```python
from build123d import *

# Parameters (mm, degrees)
LEVER_PLATE_16MM_DEPTH     = 16
HUB_FRONT_SKETCH_35_R      = 17.5
HUB_FRONT_BOSS_35X13_DEPTH = 13
HUB_START                  = 3
HUB_BACK_SKETCH_35_R       = 17.5
HUB_BACK_BOSS_35X3_DEPTH   = 3
KEYED_BORE_CUT_DEPTH       = 60
SLOT_RIM_A_2MM_DEPTH       = 2
SLOT_START                 = 2
SLOT_RIM_B_2MM_DEPTH       = 2


with BuildPart() as part:
    # Lever Profile Sketch → Lever Plate 16mm (new body)
    with BuildSketch(Plane.XY):
        with BuildLine():
            ThreePointArc((101.261586429, -17.5), (112.844778282, -11.952124129), (117.545415365, 0))
            ThreePointArc((117.545415365, 0), (113.540152463, 30.422992161), (101.797315804, 58.772707682))
            ThreePointArc((101.797315804, 58.772707682), (88.2863604, 67.464431009), (73.363703567, 61.514113087))
            ThreePointArc((73.363703567, 61.514113087), (37.333335855, 34.13389002), (-4.513207912, 16.9080145))
            ThreePointArc((-4.513207912, 16.9080145), (-17.351372478, -2.275933462), (0, -17.5))
            Line((0, -17.5), (101.261586429, -17.5))
        make_face()
        with BuildLine():
            ThreePointArc((71.407764953, 41.227292318), (79.645012795, 21.34081686), (82.454584635, 0))
            ThreePointArc((82.454584635, 0), (83.56318735, -6.137816406), (86.74890192, -11.5))
            Line((86.74890192, -11.5), (42.586205582, -11.5))
            ThreePointArc((42.586205582, -11.5), (23.157647429, 3.753303456), (33.364058597, 26.246887192))
            ThreePointArc((33.364058597, 26.246887192), (51.952476434, 37.375508628), (69.069413247, 50.656546497))
            ThreePointArc((69.069413247, 50.656546497), (69.572959936, 45.776850669), (71.407764953, 41.227292318))
        make_face(mode=Mode.SUBTRACT)
        with BuildLine():
            ThreePointArc((91.25, 0), (88.140731649, 23.617237866), (79.024818095, 45.625))
            ThreePointArc((79.024818095, 45.625), (82.227540378, 57.577722283), (94.180262662, 54.375))
            ThreePointArc((94.180262662, 54.375), (105.044433609, 28.146571155), (108.75, 0))
            ThreePointArc((108.75, 0), (100, -8.75), (91.25, 0))
        make_face(mode=Mode.SUBTRACT)
    extrude(amount=LEVER_PLATE_16MM_DEPTH)

    # Hub Front Sketch Ø35 → Hub Front Boss Ø35x13 (add)
    with BuildSketch(Plane.XY.offset(16)):
        with Locations(Location((0, 0, 0), (0, 0, 104.94534936))):
            Circle(HUB_FRONT_SKETCH_35_R)
    extrude(amount=HUB_FRONT_BOSS_35X13_DEPTH)

    # Hub Back Sketch Ø35 → Hub Back Boss Ø35x3 (add)
    with BuildSketch(Plane(origin=(0, 0, 0), x_dir=(-1, 0, 0), z_dir=(0, 0, -1)).offset(HUB_START)):
        Circle(HUB_BACK_SKETCH_35_R)
    extrude(amount=-HUB_BACK_BOSS_35X3_DEPTH)

    # Keyed Bore Sketch → Keyed Bore Cut (cut)
    with BuildSketch(Plane.XY.offset(29)):
        with BuildLine():
            ThreePointArc((-10.583005244, -3), (1.514421063, -10.895252583), (11, 0))
            Line((11, 0), (-13.5, 0))
            Line((-13.5, 0), (-13.5, -3))
            Line((-13.5, -3), (-10.583005244, -3))
        make_face()
        with BuildLine():
            Line((-13.5, 0), (11, 0))
            ThreePointArc((11, 0), (1.514421063, 10.895252583), (-10.583005244, 3))
            Line((-10.583005244, 3), (-13.5, 3))
            Line((-13.5, 3), (-13.5, 0))
        make_face()
    extrude(amount=-KEYED_BORE_CUT_DEPTH, mode=Mode.SUBTRACT)

    # Slot Rim Sketch A → Slot Rim A 2mm (add)
    with BuildSketch(Plane.XY.offset(16)):
        with BuildLine():
            ThreePointArc((117.545415365, 0), (113.540152463, 30.422992161), (101.797315804, 58.772707682))
            ThreePointArc((101.797315804, 58.772707682), (77.829832696, 65.194775426), (71.407764953, 41.227292318))
            ThreePointArc((71.407764953, 41.227292318), (79.645012795, 21.34081686), (82.454584635, 0))
            ThreePointArc((82.454584635, 0), (100, -17.545415365), (117.545415365, 0))
        make_face()
        with BuildLine():
            ThreePointArc((108.75, 0), (105.044433609, 28.146571155), (94.180262662, 54.375))
            ThreePointArc((94.180262662, 54.375), (82.227540378, 57.577722283), (79.024818095, 45.625))
            ThreePointArc((79.024818095, 45.625), (88.140731649, 23.617237866), (91.25, 0))
            ThreePointArc((91.25, 0), (100, -8.75), (108.75, 0))
        make_face(mode=Mode.SUBTRACT)
    extrude(amount=SLOT_RIM_A_2MM_DEPTH)

    # Slot Rim Sketch B → Slot Rim B 2mm (add)
    with BuildSketch(Plane(origin=(0, 0, 0), x_dir=(-1, 0, 0), z_dir=(0, 0, -1)).offset(SLOT_START)):
        with BuildLine():
            ThreePointArc((-101.797315804, 58.772707682), (-113.540152463, 30.422992161), (-117.545415365, 0))
            ThreePointArc((-117.545415365, 0), (-100, -17.545415365), (-82.454584635, 0))
            ThreePointArc((-82.454584635, 0), (-79.645012795, 21.34081686), (-71.407764953, 41.227292318))
            ThreePointArc((-71.407764953, 41.227292318), (-77.829832696, 65.194775426), (-101.797315804, 58.772707682))
        make_face()
        with BuildLine():
            ThreePointArc((-94.180262662, 54.375), (-105.044433609, 28.146571155), (-108.75, 0))
            ThreePointArc((-108.75, 0), (-100, -8.75), (-91.25, 0))
            ThreePointArc((-91.25, 0), (-88.140731649, 23.617237866), (-79.024818095, 45.625))
            ThreePointArc((-79.024818095, 45.625), (-82.227540378, 57.577722283), (-94.180262662, 54.375))
        make_face(mode=Mode.SUBTRACT)
    extrude(amount=-SLOT_RIM_B_2MM_DEPTH)


solid = part.part
```
Input: part model. Units: mm. Frame: model coordinates. A direction names the side the tool comes from. Coordinates: 2 decimals unless noted, no trailing zeros. Write each loop counter-clockwise with the first axis right and the second up, starting at its lowest first coordinate (ties: lowest second). Pieces come first, ordered by that corner, then holes. Notation, with made-up numbers: (64.5, 67.5) -> (96.5, 67.5) arc R4 cw to (96.5, 72.5) -> close; hole circle Ø9 at (9, -30.75). An arc over 180 degrees is marked (long way). Answer as a JSON object with one key per item and string values.
1. Section D-D on y = -4.5. Return the cut outline in (x, z), then the cut area to 3 significant figures.
Result set:
{"outline": "(-16.91, -3) -> (-10.04, -3) -> (-10.04, 29) -> (-16.91, 29) -> close; (10.04, -3) -> (16.91, -3) -> (16.91, 0) -> (27.39, 0) -> (27.39, 16) -> (16.91, 16) -> (16.91, 29) -> (10.04, 29) -> close; (83.04, -2) -> (92.5, -2) -> (92.5, 18) -> (83.04, 18) -> close; (107.5, -2) -> (116.96, -2) -> (116.96, 18) -> (107.5, 18) -> close", "area": "986 mm2"}
2. Section B-B on y = 48. Return the cut outline in (x, z).
Result set:
{"outline": "(57.98, 0) -> (65.97, 0) -> (65.97, 16) -> (57.98, 16) -> close; (69.17, -2) -> (78.08, -2) -> (78.08, 18) -> (69.17, 18) -> close; (97.58, -2) -> (107.3, -2) -> (107.3, 18) -> (97.58, 18) -> close"}
3. Section C-C on x = 41. Return the cut outline in (y, z).
Result set:
{"outline": "(-17.5, 0) -> (-11.44, 0) -> (-11.44, 16) -> (-17.5, 16) -> close; (30.45, 0) -> (36.29, 0) -> (36.29, 16) -> (30.45, 16) -> close"}
4. First-contact query: P1, Ø2, axis at y = 14.5, z = 22.5, coming from the -X side; P2, Ø13, axis at x = 75, z = 8.5, coming from the +Y side; P3, Ø4, axis at y = 10, z = 15, coming from the -X side. Flat tips, straight axial feed; report the tip coordinate or a pass-through.
Result set:
{"P1": "stops at x = -11.14", "P2": "stops at y = 66.79", "P3": "stops at x = -15.56"}
5. Access query for faces 1 (the face through (-12, 3, 13)), 2 (the face through (88, 16, 18)), 3 (the face through (24, -1, 0)), 4 (the face through (113.428, 30.839, 7.86)). Directions: +Z, -Z, +X, -X, +Y, -Y. A direction counts if a zero-diameter tool reaches every point of the face in a straight line with its end or side. Return the directions, or none.
Result set:
{"face 1": "+Z, -Z", "face 2": "+Z, +X, +Y, -Y", "face 3": "-Z", "face 4": "+Z, -Z, +X, +Y"}
6. Mould query, pull axis X, two halves, no side actions, for faces 5 (the face through (24, -1, 16)), 6 (the face through (37.88, 34.45, 7.89)), 7 (the face through (88, 16, -2)), 8 (the face through (51.702, 37.204, 7.888)). Classes: released by +X, released by -X, zero draft, split by the parting line, or undercut.
Result set:
{"face 5": "undercut", "face 6": "released by -X", "face 7": "zero draft", "face 8": "undercut"}
7. Material intervals for line 1 (X direction, y = -0.5, z = 21); line 2 (X direction, y = 46.5, z = 1.5); line 3 (X direction, y = -2, z = -1), sorted ascending. Write a range as from..to.
Result set:
{"line 1": "x = -17.49..-13.5, 10.99..17.49", "line 2": "x = 56.03..64.16, 69.41..78.58, 98.31..107.96", "line 3": "x = -17.39..-13.5, 10.82..17.39, 82.57..91.48, 108.52..117.43"}
8. Section A-A on z = 10. Return the cut outline in (x, y) (3 decimals).
Result set:
{"outline": "(-4.513, 16.908) arc R17.5 ccw to (0, -17.5) -> (101.262, -17.5) arc R17.545 ccw to (117.545, 0) arc R117.545 ccw to (101.797, 58.773) arc R17.545 ccw to (73.364, 61.514) arc R175 cw to start; hole (-13.5, -3) -> (-10.583, -3) arc R11 ccw (long way) to (-10.583, 3) -> (-13.5, 3) -> close; hole (33.364, 26.247) arc R20 ccw to (42.586, -11.5) -> (86.749, -11.5) arc R17.545 cw to (82.455, 0) arc R82.455 ccw to (71.408, 41.227) arc R17.545 cw to (69.069, 50.657) arc R180.022 cw to start; hole (79.025, 45.625) arc R91.25 cw to (91.25, 0) arc R8.75 ccw to (108.75, 0) arc R108.75 ccw to (94.18, 54.375) arc R8.75 ccw to start"}
